The figure shows three views and two pictorial views of one solid part (mm, origin at its lowest corner). Answer the questions. Give positions to 0.01 mm unless a question says otherwise; leave off trailing zeros. Write each loop counter-clockwise with the first axis right and the second up, starting at its lowest first coordinate (ties: lowest second). Pieces come first, ordered by that corner, then holes. Notation, with made-up numbers: M 66.25,2.5 L 81.25,2.5 A19 cw 81.25,19.5 Z; hole C 43.25,5 d8. An arc over 180 degrees is marked long. Return JSON: item names as keys, results as strings.
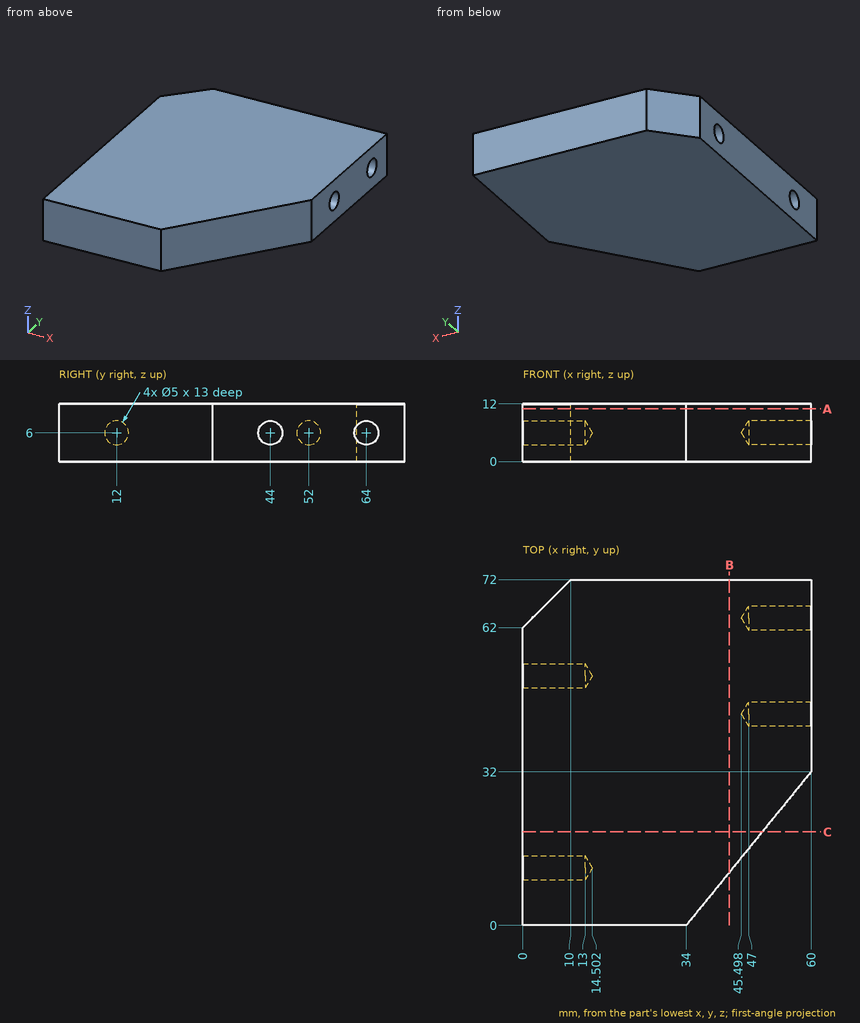
Item 1: A cutting plane is placed at A-A, the plane z = 11. Write down the section's boundary in (x, y).
Geometry results:
{"outline": "M 0,0 L 34,0 L 60,32 L 60,72 L 10,72 L 0,62 Z"}
Item 2: Find the intervals of material crossed by line 1 (Z direction, x = 3, y = 52); line 2 (Y direction, x = 56.25, z = 6) (1 decimal); line 3 (Y direction, x = 55.5, z = 6), in increasing order.
Geometry results:
{"line 1": "z = 0 to 3.5, 8.5 to 12", "line 2": "y = 27.4 to 41.5, 46.5 to 61.5, 66.5 to 72", "line 3": "y = 26.46 to 41.5, 46.5 to 61.5, 66.5 to 72"}
Item 3: Given pin 1 Ø1.5 at (x, z) = (7.5, 2.5) entering from +Y; pin 2 Ø8 at (x, y) = (30.5, 58) entering from -Z, each flat-ended and moving along its own axis, determine where each tip first touches the part or whether it passes through.
Geometry results:
{"pin 1": "stops at y = 70.25", "pin 2": "stops at z = 0"}
Item 4: A cutting plane is placed at C-C, the plane y = 19.5. Write down the section's boundary in (x, z).
Geometry results:
{"outline": "M 0,0 L 49.84,0 L 49.84,12 L 0,12 Z"}
Item 5: A cutting plane is placed at B-B, the plane x = 43. Write down the section's boundary in (y, z), plus the area to 3 significant figures.
Geometry results:
{"outline": "M 11.08,0 L 72,0 L 72,12 L 11.08,12 Z", "area": "731 mm2"}
